Part model, mm, in its own coordinate system. A direction names the side the tool comes from. Coordinates: 2 decimals unless noted, no trailing zeros. Loops run counter-clockwise (first coordinate to the right, second up) from the corner with the lowest first, then second, coordinate; pieces in that order, holes last. Notation, with made-up numbers: (-4.75, -23) -> (10.25, -23) arc R18 ccw to (10.25, -3) -> close; hole circle Ø9 at (15, 62.25). An arc over 180 degrees is marked (long way). Use one line per item in the form item = value. Start each with the question number.
(1) 3-axis set-ups, long thin cutter, end or side, ignore diameter. For faces 5 (the flat face through (-2, 1.5, -127)), 6 (the cylindrical face through (-22.66, 10.65, -15.42)), 7 (the flat face through (-2, 14, -3)): which of +Z, -Z, +X, -X, +Y, -Y reach the whole face in a straight line?
(2) Band-saw the part on B-B on z = 123. Give the cut face in (x, y), then the cut area to 4 significant figures.
(3) Pin check, flat tips, straight feed: P1, Ø12.5, axis at x = 19, z = 133, coming from the -Y side; P2, Ø7, axis at x = 62, z = -26, coming from the +Y side. Stop position of each tip, or through.
(4) Drill centre lines: L1, parallel to Z at x = -16.5, y = 13.25; L2, parallel to X at y = 9.75, z = -20.5; L3, parallel to Y at x = 33.5, z = -135.5. Where is each one in solid material? Low to high. Write a range as [from, to].
(5) Mould opens along Z. For faces 1 (the flat face through (-2, 7, 220)), 2 (the cylindrical face through (-1.66, 10.65, 25.58)), 3 (the flat face through (-23, 7.2, -18)), 4 (the flat face through (-2, 0, -185)) say: +Z half, -Z half, draft (parallel to the pull), parting line (faces both ways), or undercut.
(6) Band-saw the part on A-A on x = -96.5. Give the cut face in (y, z), then the cut area to 3 significant figures.
```python
from build123d import *

# Parameters (mm, degrees)
SKETCH_1_W                = 270
SKETCH_1_H                = 440
EXTRUDE_1_DEPTH           = 14
SKETCH_2_W                = 270
SKETCH_2_H                = 42
CUT_EXTRUDE_1_DEPTH       = 1.5
HOLE_WIZARD_1_D           = 6.6
HOLE_WIZARD_1_CBORE_D     = 11
HOLE_WIZARD_1_CBORE_DEPTH = 6.8
SKETCH_4_W                = 14.5
SKETCH_4_H                = 180
CUT_EXTRUDE_2_DEPTH       = 1.5
CUT_EXTRUDE_3_REACH       = 260.498
SKETCH_5_R                = 2.5


with BuildPart() as part:
    # 草图1 → 凸台-拉伸1 (new body)
    with BuildSketch(Plane(origin=(0, 0, 0), x_dir=(1, 0, 0), z_dir=(0, 1, 0))):
        Rectangle(SKETCH_1_W, SKETCH_1_H)
    extrude(amount=EXTRUDE_1_DEPTH)

    # 草图2 → 切除-拉伸1 (cut)
    with BuildSketch(Plane.XZ):
        with Locations((0, 127)):
            Rectangle(SKETCH_2_W, SKETCH_2_H)
        with Locations((0, -127)):
            Rectangle(SKETCH_2_W, SKETCH_2_H)
    extrude(amount=-CUT_EXTRUDE_1_DEPTH, mode=Mode.SUBTRACT)

    # 打孔尺寸(%根据)内六角圆柱头螺钉的类型1 (through all)
    with Locations(Plane(origin=(-20.55, 14, 20.5), x_dir=(0, 0, 1), z_dir=(0, 1, 0))):
        with Locations((0, 0), (-41, 0), (0, 21), (-41, 21)):
            CounterBoreHole(HOLE_WIZARD_1_D / 2, HOLE_WIZARD_1_CBORE_D / 2, HOLE_WIZARD_1_CBORE_DEPTH)

    # 草图4 → 切除-拉伸2 (cut)
    with BuildSketch(Plane(origin=(0, 14, 0), x_dir=(1, 0, 0), z_dir=(0, 1, 0))):
        with Locations((62.75, 0)):
            Rectangle(SKETCH_4_W, SKETCH_4_H)
    extrude(amount=-CUT_EXTRUDE_2_DEPTH, mode=Mode.SUBTRACT)

    # 草图5 → 切除-拉伸3 (cut, up to next)
    with BuildSketch(Plane(origin=(0, 14, 0), x_dir=(1, 0, 0), z_dir=(0, 1, 0)), mode=Mode.PRIVATE) as cut_extrude_3_sk1:
        with Locations(Location((55.5, 90, 0), (0, 0, 270))):
            Circle(SKETCH_5_R)
    cut_extrude_3_tool1 = extrude(cut_extrude_3_sk1.sketch, amount=-CUT_EXTRUDE_3_REACH, mode=Mode.PRIVATE) & part.part
    # 草图5 → 切除-拉伸3 (cut, up to next)
    with BuildSketch(Plane(origin=(0, 14, 0), x_dir=(1, 0, 0), z_dir=(0, 1, 0)), mode=Mode.PRIVATE) as cut_extrude_3_sk2:
        with Locations(Location((70, 90, 0), (0, 0, 270))):
            Circle(SKETCH_5_R)
    cut_extrude_3_tool2 = extrude(cut_extrude_3_sk2.sketch, amount=-CUT_EXTRUDE_3_REACH, mode=Mode.PRIVATE) & part.part
    # 草图5 → 切除-拉伸3 (cut, up to next)
    with BuildSketch(Plane(origin=(0, 14, 0), x_dir=(1, 0, 0), z_dir=(0, 1, 0)), mode=Mode.PRIVATE) as cut_extrude_3_sk3:
        with Locations(Location((55.5, -90, 0), (0, 0, 90))):
            Circle(SKETCH_5_R)
    cut_extrude_3_tool3 = extrude(cut_extrude_3_sk3.sketch, amount=-CUT_EXTRUDE_3_REACH, mode=Mode.PRIVATE) & part.part
    # 草图5 → 切除-拉伸3 (cut, up to next)
    with BuildSketch(Plane(origin=(0, 14, 0), x_dir=(1, 0, 0), z_dir=(0, 1, 0)), mode=Mode.PRIVATE) as cut_extrude_3_sk4:
        with Locations(Location((70, -90, 0), (0, 0, 90))):
            Circle(SKETCH_5_R)
    cut_extrude_3_tool4 = extrude(cut_extrude_3_sk4.sketch, amount=-CUT_EXTRUDE_3_REACH, mode=Mode.PRIVATE) & part.part
    add(cut_extrude_3_tool1.solids().sort_by_distance((55.5, 14, -90))[0], mode=Mode.SUBTRACT)
    add(cut_extrude_3_tool2.solids().sort_by_distance((70, 14, -90))[0], mode=Mode.SUBTRACT)
    add(cut_extrude_3_tool3.solids().sort_by_distance((55.5, 14, 90))[0], mode=Mode.SUBTRACT)
    add(cut_extrude_3_tool4.solids().sort_by_distance((70, 14, 90))[0], mode=Mode.SUBTRACT)


solid = part.part
```
A:
q1.face_5 = +X, -X, -Y
q1.face_6 = +Y
q1.face_7 = +Z, -Z, +X, -X, +Y
q2.outline = (-135, 1.5) -> (135, 1.5) -> (135, 14) -> (-135, 14) -> close
q2.area = 3,375 mm²
q3.P1 = 1.5
q3.P2 = 12.5
q4.L1 = [-220, -24.22], [-16.78, 16.78], [24.22, 220]
q4.L2 = [-135, -26.05], [-15.05, -5.05], [5.95, 135]
q4.L3 = [1.5, 14]
q5.face_1 = +Z half
q5.face_2 = undercut
q5.face_3 = undercut
q5.face_4 = draft
q6.outline = (0, -220) -> (14, -220) -> (14, 220) -> (0, 220) -> (0, 148) -> (1.5, 148) -> (1.5, 106) -> (0, 106) -> (0, -106) -> (1.5, -106) -> (1.5, -148) -> (0, -148) -> close
q6.area = 6,030 mm²
